Here's the drawing with two shaded views (mm, measured from the low corner). I have some questions. A direction names the side the tool comes from. Coordinates: 2 decimals unless noted, no trailing zeros. Order: outer loops, then holes, each group sorted by start corner. A loop starts at its lowest first (then second) coordinate and runs counter-clockwise, first axis right, second up. Notation, with made-up numbers: (-33, 25) -> (2, 25) arc R17 ccw to (2, 48) -> close; hole circle Ø2 at (4.5, 11). An arc over 180 degrees is marked (long way). Answer as a JSON object with one key per item and string values. Group by question number.
(1) Which directions (+Z, -Z, +X, -X, +Y, -Y) give clear straight access to the entire face, cutting with the end or side of a thin tool? Please do the marked faces 1 and 2.
(2) I want a section at C-C, the plane z = 14.5. List the corners of the cut face in (x, y) for me.
(3) For pin 1 (8 mm diameter, centred on x = 67.5, z = 24, fed in from +Y); pin 2 (10 mm diameter, centred on x = 71, y = 60.5, fed in from +Z); pin 3 (1.5 mm diameter, centred on y = 20.5, z = 31.5, fed in from -X), each with a flat end and sliding along its axis, tell me the tip position at first contact or that it passes through.
(4) I want a section at A-A, the plane x = 40. List the corners of the cut face in (y, z) for me, plus the area to 3 significant figures.
(5) I want a section at D-D, the plane z = 48. List the corners of the cut face in (x, y) for me.
(6) I want a section at B-B, the plane y = 32. List the corners of the cut face in (x, z) for me.
(7) I need wall thicknesses on line 1 (Y direction, x = 40, z = 38); line 2 (Y direction, x = 40, z = 19); line 3 (Z direction, x = 47.5, y = 7). Which ranges of each line are inside material? Lowest first, please.
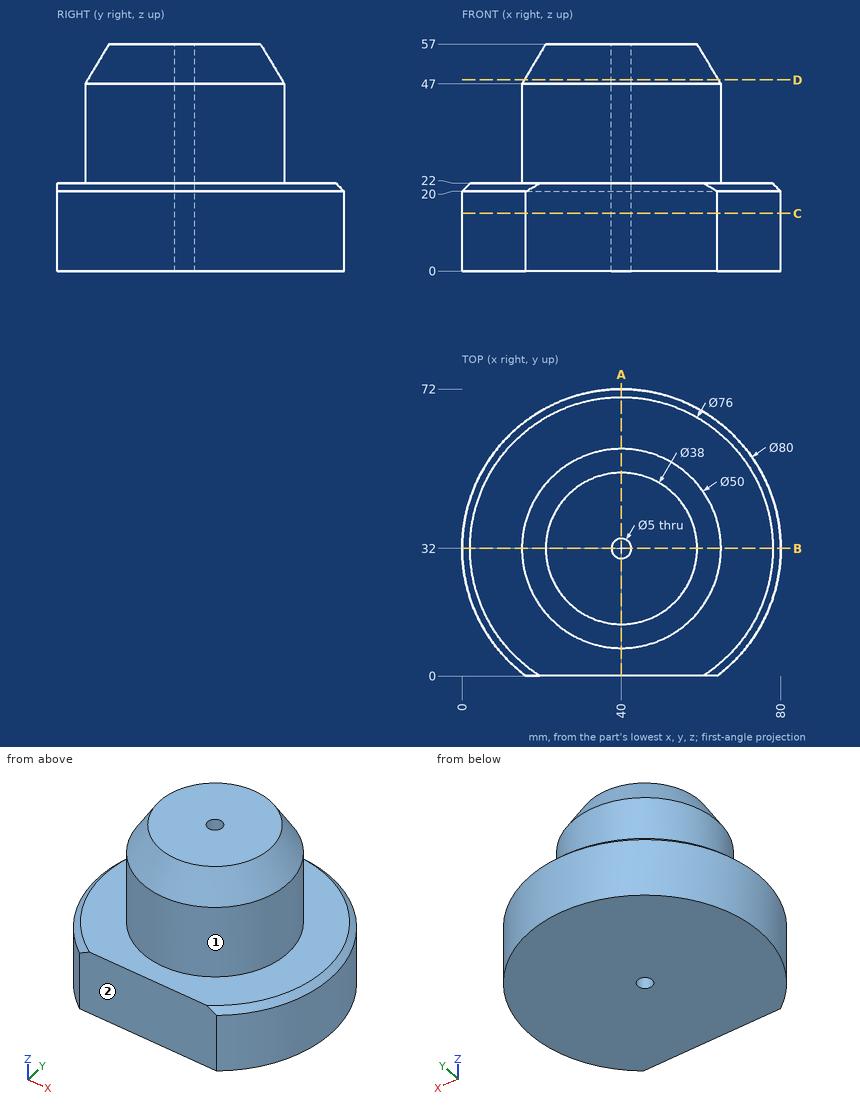
Computed values:
{
 "1": {"face 1": "+Z", "face 2": "+Z, -Z, +X, -X, -Y"},
 "2": {"outline": "(16, 0) -> (64, 0) arc R40 ccw (long way) to start; hole circle Ø5 at (40, 32)"},
 "3": {"pin 1": "stops at y = 62.13", "pin 2": "stops at z = 22", "pin 3": "stops at x = 17.43"},
 "4": {"outline": "(0, 0) -> (29.5, 0) -> (29.5, 57) -> (13, 57) -> (7, 47) -> (7, 22) -> (0, 22) -> close; (34.5, 0) -> (72, 0) -> (72, 20) -> (70, 22) -> (57, 22) -> (57, 47) -> (51, 57) -> (34.5, 57) -> close", "area": "2,990 mm2"},
 "5": {"outline": "circle Ø48.8 at (40, 32); hole circle Ø5 at (40, 32)"},
 "6": {"outline": "(0, 0) -> (37.5, 0) -> (37.5, 57) -> (21, 57) -> (15, 47) -> (15, 22) -> (2, 22) -> (0, 20) -> close; (42.5, 0) -> (80, 0) -> (80, 20) -> (78, 22) -> (65, 22) -> (65, 47) -> (59, 57) -> (42.5, 57) -> close"},
 "7": {"line 1": "y = 7 to 29.5, 34.5 to 57", "line 2": "y = 0 to 29.5, 34.5 to 72", "line 3": "z = 0 to 22"}
}
